The model under review builds one solid part; all positions refer to its coordinate system, in mm. Face numbers are marked on the shaded views. A direction names the side the tool comes from. Round coordinates to 2 decimals unless told otherwise and drop trailing zeros. Loops run counter-clockwise (first coordinate to the right, second up) from the corner with the lowest first, then second, coordinate; pieces in that order, holes last. Notation, with made-up numbers: M 75,77.25 L 110,77.25 A36 ccw 110,115.25 Z; hole C 43.25,20.5 d4. An arc over 180 degrees is marked long. Answer as a JSON object with one key per item and string values. Group by question number.
Item 1: The part is to be moulded in two halves that separate along Y. For the marked faces 4, 5, 6 and 7, say which applies: +Y half, -Y half, draft (parallel to the pull), parting line (faces both ways), or undercut.
Item 2: Consider section B-B (x = 26.5). Give the boundary of the cut face in (y, z), and give its area (3 significant figures).
Item 3: Tool access review of the marked faces 1, 2 and 3: name each direction out of +Z, -Z, +X, -X, +Y, -Y from which nothing blocks a thin tool from reaching the whole face with its end or side.
Item 4: Consider section D-D (x = 15.5). Give the boundary of the cut face in (y, z), and give its area (3 significant figures).
Item 5: Insertion check: P1, Ø2, axis at y = 0, z = 30, coming from the -X side; P2, Ø8, axis at x = 17.5, y = -20.5, coming from the -Z side; P3, Ø3.5, axis at x = 3.5, y = -5, coming from the +Z side. Each pin has a flat end and moves straight along its axis. Give the tip position at first contact, or say it passes through.
Item 6: To check wall thickness, follow line 1 (Y direction, x = 6.5, z = 26.25); line 2 (X direction, y = 13, z = 20); line 3 (Y direction, x = 38.25, z = 0). State the ranges of each line that lie inside material, in increasing order.
Item 7: Consider section A-A (x = 3.5). Give the boundary of the cut face in (y, z).
Item 8: Consider section C-C (x = 37). Give the boundary of the cut face in (y, z).
```python
from build123d import *

# Parameters (mm, degrees)
SKETCH1_R             = 35
BOSS_EXTRUDE1_DEPTH   = 20
SKETCH2_R             = 35
BOSS_EXTRUDE2_DEPTH   = 10
SKETCH3_R             = 24.95
BOSS_EXTRUDE3_DEPTH   = 12
SKETCH4_R             = 21
CUT_EXTRUDE1_DEPTH    = 12
SKETCH5_R             = 19
CUT_EXTRUDE2_DEPTH    = 18
SKETCH6_R             = 21
CUT_EXTRUDE3_DEPTH    = 28
CIRPATTERN1_COUNT     = 4
SKETCH9_W             = 82.925750659
SKETCH9_H             = 79.628478102
CUT_EXTRUDE4_DEPTH    = 12
M4_TAPPED_HOLE3_D     = 3.3
M4_TAPPED_HOLE3_DEPTH = 10.1
M4_TAPPED_HOLE3_TIP   = 0.991420021
CHAMFER1_SIZE         = 1


with BuildPart() as part:
    # Sketch1 → Boss-Extrude1 (new body)
    with BuildSketch(Plane(origin=(0, 0, 0), x_dir=(0, 0, -1), z_dir=(1, 0, 0))):
        Circle(SKETCH1_R)
    extrude(amount=BOSS_EXTRUDE1_DEPTH)

    # Sketch2 → Boss-Extrude2 (add)
    with BuildSketch(Plane(origin=(20, 0, 0), x_dir=(0, 0, -1), z_dir=(1, 0, 0))):
        Circle(SKETCH2_R)
    extrude(amount=BOSS_EXTRUDE2_DEPTH)

    # Sketch3 → Boss-Extrude3 (add)
    with BuildSketch(Plane(origin=(30, 0, 0), x_dir=(0, 0, -1), z_dir=(1, 0, 0))):
        Circle(SKETCH3_R)
    extrude(amount=BOSS_EXTRUDE3_DEPTH)

    # Sketch4 → Cut-Extrude1 (cut)
    with BuildSketch(Plane.ZY):
        Circle(SKETCH4_R)
    extrude(amount=-CUT_EXTRUDE1_DEPTH, mode=Mode.SUBTRACT)

    # Sketch5 → Cut-Extrude2 (cut)
    with BuildSketch(Plane.ZY.offset(-12)):
        Circle(SKETCH5_R)
    extrude(amount=-CUT_EXTRUDE2_DEPTH, mode=Mode.SUBTRACT)

    # Sketch6 → Cut-Extrude3 (cut)
    with BuildSketch(Plane.ZY.offset(-30)):
        Circle(SKETCH6_R)
    extrude(amount=-CUT_EXTRUDE3_DEPTH, mode=Mode.SUBTRACT)

    # Sketch7 → M4 Tapped Hole2 (revolve, cut)
    with BuildSketch(Plane(origin=(30, 0, -30), x_dir=(0, 0, -1), z_dir=(0, 1, 0))):
        Polygon((0, 0), (0, 11.091420021), (1.65, 10.1), (1.65, 0), align=None)
    m4_tapped_hole2 = revolve(axis=Axis((36.35, 0, -30), (-1, 0, 0)), mode=Mode.SUBTRACT)

    # CirPattern1: M4 Tapped Hole2 ×4 about axis
    cirpattern1_axis = Axis((0, 0, 0), (1, 0, 0))
    for i in range(1, CIRPATTERN1_COUNT):
        add(m4_tapped_hole2.rotate(cirpattern1_axis, i * 360 / CIRPATTERN1_COUNT), mode=Mode.SUBTRACT)

    # Sketch9 → Cut-Extrude4 (cut)
    with BuildSketch(Plane.ZY):
        with Locations((69.46287533, 0)):
            Rectangle(SKETCH9_W, SKETCH9_H)
    extrude(amount=-CUT_EXTRUDE4_DEPTH, mode=Mode.SUBTRACT)

    # M4 Tapped Hole3
    with Locations(Plane.XY.offset(28)):
        with Locations((6.5, 13), (6.5, -13)):
            Hole(M4_TAPPED_HOLE3_D / 2, depth=M4_TAPPED_HOLE3_DEPTH)
            with Locations((0, 0, -(M4_TAPPED_HOLE3_DEPTH + M4_TAPPED_HOLE3_TIP / 2))):  # 118° drill point
                Cone(0, M4_TAPPED_HOLE3_D / 2, M4_TAPPED_HOLE3_TIP, mode=Mode.SUBTRACT)

    # Chamfer1
    chamfer1_edges = [part.edges().sort_by_distance(p)[0] for p in [
        (42, 0, 24.95),
        (0, 0, -21),
        (42, 0, -21),
        (0, 33.203915432, -11.067971811),
        (30, 0, 35),
    ]]
    chamfer(chamfer1_edges, length=CHAMFER1_SIZE)


solid = part.part
```
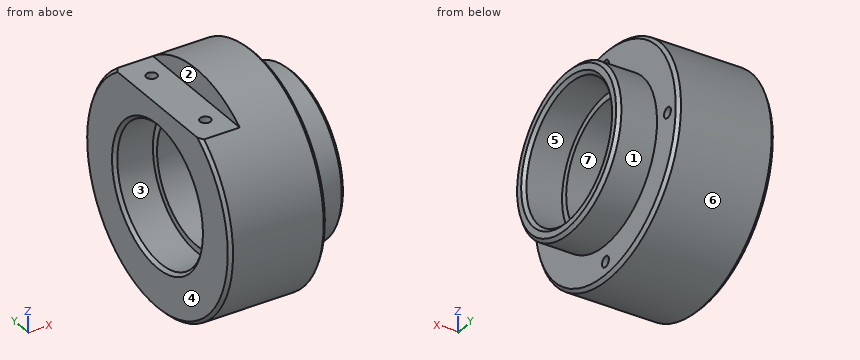
Geometry results:
{
 "1": {"face 4": "draft", "face 5": "undercut", "face 6": "parting line", "face 7": "undercut"},
 "2": {"outline": "C 0,0 d70; hole C -30,0 d3.3; hole C 0,0 d38; hole C 0,-30 d3.3; hole C 0,30 d3.3; hole C 30,0 d3.3", "area": "2,680 mm^2"},
 "3": {"face 1": "+X", "face 2": "+Z, -X, +Y, -Y", "face 3": "-X"},
 "4": {"outline": "C 0,0 d70; hole C 0,0 d38", "area": "2,710 mm^2"},
 "5": {"P1": "stops at x = 12", "P2": "stops at z = -30.87", "P3": "stops at z = 28"},
 "6": {"line 1": "y = -23.15 to -14.65, -11.35 to 11.35, 14.65 to 23.15", "line 2": "x = 0 to 4.85, 8.15 to 42", "line 3": "y = -24.95 to -21, 21 to 24.95"},
 "7": {"outline": "M -21,28 A35 ccw long 21,28 Z; hole C 0,0 d42"},
 "8": {"outline": "C 0,0 d49.9; hole C 0,0 d42"}
}
